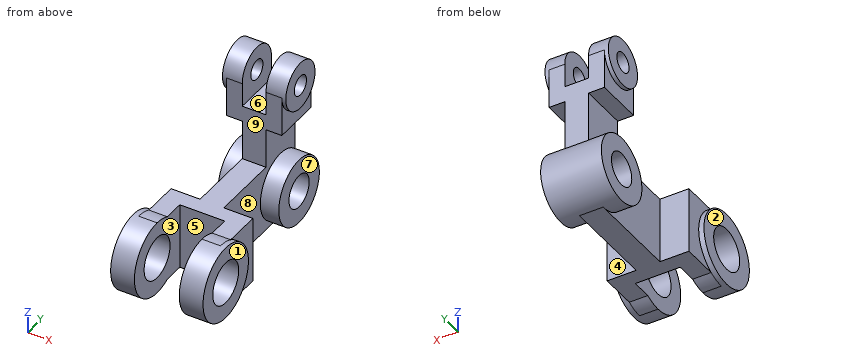
from build123d import *

# Parameters (mm, degrees)
CLEVIS_EYE_A_SKETCH_R        = 28
CLEVIS_EYE_A_56_DEPTH        = 18
CLEVIS_EYE_B_SKETCH_R        = 28
CLEVIS_EYE_B_56_DEPTH        = 18
CLEVIS_BORE_SKETCH_R         = 16
CLEVIS_BORE_DEPTH            = 95
LINK_WEB_DEPTH               = 28
WEB_GUSSET_1_DEPTH           = 14
WEB_START                    = -14
WEB_GUSSET_2_DEPTH           = 14
WEB_SLOT_CUT_DEPTH           = 74
LOWER_FORK_BLOCK_SKETCH_W    = 18
LOWER_FORK_BLOCK_SKETCH_H    = 70
LOWER_FORK_BLOCK_DEPTH       = 50
LOWER_FORK_EYE_DEPTH         = 14
LOWER_FORK_EYE_DEPTH_BACK    = 32
LOWER_FORK_EYE_SKETCH_R      = 25
UPPER_FORK_PROFILE_DEPTH     = 18
UPPER_FORK_EYE_36_DEPTH      = 3
UPPER_FORK_EYE_36_DEPTH_BACK = 12
UPPER_FORK_EYE_SKETCH_36_R   = 18
UPPER_FORK_HUB_SKETCH_R      = 18
UPPER_FORK_HUB_DEPTH         = 15
UPPER_FORK_PIN_BORE_SKETCH_R = 7.5
UPPER_FORK_PIN_BORE_DEPTH    = 152
LOWER_FORK_PIN_BORE_SKETCH_R = 12.5
LOWER_FORK_PIN_BORE_DEPTH    = 152


with BuildPart() as part:
    # Clevis Eye A Sketch → Clevis Eye A Ø56 (new body)
    with BuildSketch(Plane(origin=(0, 0, 0), x_dir=(0, 0, -1), z_dir=(1, 0, 0))):
        Circle(CLEVIS_EYE_A_SKETCH_R)
    extrude(amount=-CLEVIS_EYE_A_56_DEPTH)


with BuildPart() as body_2:
    # Clevis Eye B Sketch → Clevis Eye B Ø56 (new body)
    with BuildSketch(Plane.ZY.offset(52)):
        with Locations(Location((0, 0, 0), (0, 0, 180))):
            Circle(CLEVIS_EYE_B_SKETCH_R)
    extrude(amount=CLEVIS_EYE_B_56_DEPTH)


with BuildPart() as clevis_bore_tool:
    # Clevis Bore Sketch → Clevis Bore (new body)
    with BuildSketch(Plane(origin=(0, 0, 0), x_dir=(0, 0, -1), z_dir=(1, 0, 0))):
        Circle(CLEVIS_BORE_SKETCH_R)
    extrude(amount=-CLEVIS_BORE_DEPTH)


with BuildPart() as part_1:
    add(part.part)

    # Clevis Bore: cut by clevis_bore_tool
    add(clevis_bore_tool.part, mode=Mode.SUBTRACT)



with BuildPart() as body_2_1:
    add(body_2.part)

    # Clevis Bore: cut by clevis_bore_tool
    add(clevis_bore_tool.part, mode=Mode.SUBTRACT)


with BuildPart() as part_2:
    add(part_1.part)

    add(body_2_1.part)  # Link Web merges body 2
    # Link Web Sketch → Link Web (add, symmetric)
    with BuildSketch(Plane.XY):
        Polygon((-66, 40), (-66, 16), (-52, 16), (-52, 26), (-52, 28), (-18, 28), (-18, 26), (-18, 16), (-4, 16), (-4, 40), align=None)
    extrude(amount=LINK_WEB_DEPTH, both=True)

    # Web Gusset 1 Sketch → Web Gusset 1 (add)
    with BuildSketch(Plane(origin=(-4, 0, 0), x_dir=(0, 0, -1), z_dir=(1, 0, 0))):
        with BuildLine():
            Line((-28, 16), (-28, 0))
            ThreePointArc((-28, 0), (-26.71508, 8.384777), (-22.978251, 16))
            Line((-22.978251, 16), (-28, 16))
        make_face()
        with BuildLine():
            Line((28, 16), (28, 0))
            ThreePointArc((28, 0), (26.71508, 8.384777), (22.978251, 16))
            Line((22.978251, 16), (28, 16))
        make_face()
    extrude(amount=-WEB_GUSSET_1_DEPTH)

    # Web Gusset 2 Sketch → Web Gusset 2 (add)
    with BuildSketch(Plane.ZY.offset(66).offset(WEB_START)):
        with BuildLine():
            Line((28, 16), (28, 0))
            ThreePointArc((28, 0), (26.71508, 8.384777), (22.978251, 16))
            Line((22.978251, 16), (28, 16))
        make_face()
        with BuildLine():
            Line((-28, 0), (-28, 16))
            Line((-28, 16), (-22.978251, 16))
            ThreePointArc((-22.978251, 16), (-26.71508, 8.384777), (-28, 0))
        make_face()
    extrude(amount=WEB_GUSSET_2_DEPTH)

    # Web Slot Sketch → Web Slot Cut (cut)
    with BuildSketch(Plane(origin=(-4, 0, 0), x_dir=(0, 0, -1), z_dir=(1, 0, 0))):
        with BuildLine():
            Line((-25, 12.60952), (-25, 40))
            Line((-25, 40), (-28, 40))
            Line((-28, 40), (-28, 0))
            ThreePointArc((-28, 0), (-27.239677, 6.480741), (-25, 12.60952))
        make_face()
        with BuildLine():
            Line((28, 40), (25, 40))
            Line((25, 40), (25, 12.60952))
            ThreePointArc((25, 12.60952), (27.239677, 6.480741), (28, 0))
            Line((28, 0), (28, 40))
        make_face()
    extrude(amount=-WEB_SLOT_CUT_DEPTH, mode=Mode.SUBTRACT)

    # Lower Fork Block Sketch → Lower Fork Block (add)
    with BuildSketch(Plane.XY.offset(25)):
        with Locations((-35, 75)):
            Rectangle(LOWER_FORK_BLOCK_SKETCH_W, LOWER_FORK_BLOCK_SKETCH_H)
    extrude(amount=-LOWER_FORK_BLOCK_DEPTH)

    # Lower Fork Eye Sketch → Lower Fork Eye (add, two sides: drawn at the far end of the back side and taken through both)
    with BuildSketch(Plane.ZY.offset(44).offset(-LOWER_FORK_EYE_DEPTH_BACK)):
        with Locations((0, 110)):
            Circle(LOWER_FORK_EYE_SKETCH_R)
    extrude(amount=LOWER_FORK_EYE_DEPTH + LOWER_FORK_EYE_DEPTH_BACK)

    # Upper Fork Profile Sketch → Upper Fork Profile (add, symmetric)
    with BuildSketch(Plane(origin=(0, 110, 0), x_dir=(1, 0, 0), z_dir=(0, 1, 0))):
        Polygon((-26, -55), (-14, -55), (-14, -85), (-26, -85), (-26, -67), (-44, -67), (-44, -85), (-56, -85), (-56, -55), (-44, -55), (-44, 0), (-26, 0), align=None)
    extrude(amount=UPPER_FORK_PROFILE_DEPTH, both=True)

    # Upper Fork Eye Sketch Ø36 → Upper Fork Eye Ø36 (add, two sides: drawn at the far end of the back side and taken through both)
    with BuildSketch(Plane(origin=(-14, 0, 0), x_dir=(0, 0, -1), z_dir=(1, 0, 0)).offset(-UPPER_FORK_EYE_36_DEPTH_BACK)):
        with Locations((-85, 110)):
            Circle(UPPER_FORK_EYE_SKETCH_36_R)
    extrude(amount=UPPER_FORK_EYE_36_DEPTH + UPPER_FORK_EYE_36_DEPTH_BACK)

    # Upper Fork Hub Sketch → Upper Fork Hub (add)
    with BuildSketch(Plane(origin=(-44, 0, 0), x_dir=(0, 0, -1), z_dir=(1, 0, 0))):
        with Locations((-85, 110)):
            Circle(UPPER_FORK_HUB_SKETCH_R)
    extrude(amount=-UPPER_FORK_HUB_DEPTH)

    # Upper Fork Pin Bore Sketch → Upper Fork Pin Bore (cut)
    with BuildSketch(Plane(origin=(-11, 0, 0), x_dir=(0, 0, -1), z_dir=(1, 0, 0))):
        with Locations((-85, 110)):
            Circle(UPPER_FORK_PIN_BORE_SKETCH_R)
    extrude(amount=-UPPER_FORK_PIN_BORE_DEPTH, mode=Mode.SUBTRACT)

    # Lower Fork Pin Bore Sketch → Lower Fork Pin Bore (cut)
    with BuildSketch(Plane(origin=(-12, 0, 0), x_dir=(0, 0, -1), z_dir=(1, 0, 0))):
        with Locations((0, 110)):
            Circle(LOWER_FORK_PIN_BORE_SKETCH_R)
    extrude(amount=-LOWER_FORK_PIN_BORE_DEPTH, mode=Mode.SUBTRACT)


solid = part_2.part
Check sheet for the modelled part. Datum: model origin and axes. Units: mm. Face numbers are marked on the shaded views. A direction names the side the tool comes from. Give positions to 0.01 mm unless a question says otherwise; leave off trailing zeros. Order: outer loops, then holes, each group sorted by start corner. A loop starts at its lowest first (then second) coordinate and runs counter-clockwise, first axis right, second up. Notation, with made-up numbers: M 81,39.25 L 108,39.25 A33 ccw 108,76.25 Z; hole C 84.25,70 d8. An arc over 180 degrees is marked long. Answer as CSV lines item,"result". Start each with the question number.
Item 1: Cross-section at C-C on x = -6. Enter the section's corners in (y, z).
Item 2: Cross-section at D-D on y = 8. Enter the section's corners in (x, z), plus the area to 3 significant figures.
Item 3: Cross-section at B-B on z = 0. State how many separate pieces and enclosed holes the cut face has, plus the area to 3 significant figures.
Item 4: Cross-section at A-A on x = -54. Enter the section's corners in (y, z).
Item 5: Tool access check on the marked faces 5, 6, 7, 8 and 9. Record the directions out of +Z, -Z, +X, -X, +Y, -Y that give a thin tool (end or side, any length) a straight path to the whole face; none if there is none.
Item 6: Thickness scan on line 1 (Z direction, x = -3, y = 0); line 2 (Y direction, x = -8, z = 0); line 3 (X direction, y = 50, z = -10.5). Record the ranges inside material, lowest first. Write a range as [from, to].
Item 7: Gauge pin test, flat ends, axial feed: P1, Ø24, axis at x = -16.5, z = -4.5, coming from the +Y side; P2, Ø12, axis at x = -29, y = 118.5, coming from the -Z side; P3, Ø9.5, axis at x = -22.5, y = 101.5, coming from the -Z side. Record the tip position at first contact, or that the pin passes through.
Item 8: Mould release check, pull along X, two halves, no side actions. Record for the marked faces 1, 2, 3 and 4: +X half, -X half, draft (parallel to the pull), parting line (faces both ways), or undercut.
Established:
1,outline,"M 0,-28 A28 ccw 12.61,-25 L 40,-25 L 40,25 L 12.61,25 A28 ccw 0,28 A28 ccw Z; hole C 0,0 d32"
2,outline,"M -70,-26.83 L -52,-26.83 L -52,-13.86 L -70,-13.86 Z; M -70,13.86 L -52,13.86 L -52,26.83 L -70,26.83 Z; M -18,-26.83 L 0,-26.83 L 0,-13.86 L -18,-13.86 Z; M -18,13.86 L 0,13.86 L 0,26.83 L -18,26.83 Z"
2,area,"934 mm^2"
3,separate pieces,"4"
3,enclosed holes,"0"
3,area,"3,570 mm^2"
4,outline,"M 0,-28 A28 ccw 12.61,-25 L 40,-25 L 40,25 L 12.61,25 A28 ccw 0,28 A28 ccw Z; C 110,0 d50; M 92,55 L 128,55 L 128,85 A18 ccw 92,85 Z; hole C 0,0 d32; hole C 110,0 d25; hole C 110,85 d15"
5,face 5,"+Z, -Z, -Y"
5,face 6,"+Z, +Y, -Y"
5,face 7,"-Z, +X, +Y"
5,face 8,"+X"
5,face 9,"+Z, +X, -X, -Y"
6,line 1,"z = [-28, -16], [16, 28]"
6,line 2,"y = [-28, -16], [16, 40]"
6,line 3,"x = [-44, -26]"
7,P1,"stops at y = 135"
7,P2,"stops at z = -24.87"
7,P3,"stops at z = -25"
8,face 1,"+X half"
8,face 2,"-X half"
8,face 3,"undercut"
8,face 4,"draft"
